from build123d import *

# Parameters (mm, degrees)
SKETCH_1_W             = 135
SKETCH_1_H             = 100
EXTRUDE_1_DEPTH        = 12
SKETCH_2_W             = 12.5
SKETCH_2_H             = 100
EXTRUDE_2_DEPTH        = 15
SKETCH_3_W             = 30
SKETCH_3_H             = 200
CUT_EXTRUDE_1_DEPTH    = 4
SKETCH_4_W             = 60
SKETCH_4_H             = 20
CUT_EXTRUDE_2_DEPTH    = 86.330240829
FILLET_1_R             = 5
HOLE_WIZARD_M6_1_D     = 5
HOLE_WIZARD_M6_1_DEPTH = 15
HOLE_WIZARD_M6_1_TIP   = 1.502151548
HOLE_WIZARD_M5_1_D     = 4.2
HOLE_WIZARD_M5_1_DEPTH = 12.4
HOLE_WIZARD_M5_1_TIP   = 1.2618073
CHAMFER_1_SIZE         = 0.5


with BuildPart() as part:
    # 草图1 → 凸台-拉伸1 (new body)
    with BuildSketch(Plane.XY):
        Rectangle(SKETCH_1_W, SKETCH_1_H)
    extrude(amount=EXTRUDE_1_DEPTH)

    # 草图2 → 凸台-拉伸2 (add)
    with BuildSketch(Plane.XY.offset(12)):
        with Locations((-61.25, 0)):
            Rectangle(SKETCH_2_W, SKETCH_2_H)
        with Locations((61.25, 0)):
            Rectangle(SKETCH_2_W, SKETCH_2_H)
    extrude(amount=EXTRUDE_2_DEPTH)

    # 草图3 → 切除-拉伸1 (cut)
    with BuildSketch(Plane.XY.offset(12)):
        with Locations((0, 50)):
            Rectangle(SKETCH_3_W, SKETCH_3_H)
    extrude(amount=-CUT_EXTRUDE_1_DEPTH, mode=Mode.SUBTRACT)

    # 草图4 → 切除-拉伸2 (cut, through all)
    with BuildSketch(Plane.XY.offset(12)):
        with Locations((0, 40)):
            Rectangle(SKETCH_4_W, SKETCH_4_H)
    extrude(amount=-CUT_EXTRUDE_2_DEPTH, mode=Mode.SUBTRACT)

    # 圆角1
    fillet_1_edges = [part.edges().sort_by_distance(p)[0] for p in [
        (30, 30, 6),
        (-30, 30, 6),
    ]]
    fillet(fillet_1_edges, radius=FILLET_1_R)

    # M6 螺纹孔1
    with Locations(Plane(origin=(0, 50, 0), x_dir=(1, 0, 0), z_dir=(0, 1, 0))):
        with Locations((-61.5, -21), (-47.5, -6), (47.5, -6), (61.5, -21)):
            Hole(HOLE_WIZARD_M6_1_D / 2, depth=HOLE_WIZARD_M6_1_DEPTH)
            with Locations((0, 0, -(HOLE_WIZARD_M6_1_DEPTH + HOLE_WIZARD_M6_1_TIP / 2))):  # 118° drill point
                Cone(0, HOLE_WIZARD_M6_1_D / 2, HOLE_WIZARD_M6_1_TIP, mode=Mode.SUBTRACT)

    # M5 螺纹孔1
    with Locations(Plane.XY.offset(27)):
        with Locations((-61.5, 30), (-61.5, -30), (61.5, -30), (61.5, 30)):
            Hole(HOLE_WIZARD_M5_1_D / 2, depth=HOLE_WIZARD_M5_1_DEPTH)
            with Locations((0, 0, -(HOLE_WIZARD_M5_1_DEPTH + HOLE_WIZARD_M5_1_TIP / 2))):  # 118° drill point
                Cone(0, HOLE_WIZARD_M5_1_D / 2, HOLE_WIZARD_M5_1_TIP, mode=Mode.SUBTRACT)

    # 倒角1
    chamfer_1_edges = [part.edges().sort_by_distance(p)[0] for p in [
        (-35, -50, 12),
        (-55, -50, 19.5),
        (-55, 50, 19.5),
        (-67.5, 0, 27),
        (-61.25, -50, 27),
        (-55, 0, 27),
        (-61.25, 50, 27),
        (42.5, 50, 12),
        (55, 50, 19.5),
        (55, -50, 19.5),
        (61.25, 50, 27),
        (55, 0, 27),
        (61.25, -50, 27),
        (67.5, 0, 27),
        (35, -50, 12),
        (0, -50, 0),
        (-67.5, 0, 0),
        (48.75, 50, 0),
        (67.5, 0, 0),
        (-48.75, 50, 0),
        (-42.5, 50, 12),
        (-30, 50, 6),
        (30, 50, 6),
        (67.5, -50, 13.5),
        (-67.5, -50, 13.5),
        (-67.5, 50, 13.5),
        (67.5, 50, 13.5),
    ]]
    chamfer(chamfer_1_edges, length=CHAMFER_1_SIZE)


solid = part.part
Design review of the part built by this model. Coordinates are the model's own, in mm. A direction names the side the tool comes from. Coordinates: 2 decimals unless noted, no trailing zeros. Loops run counter-clockwise (first coordinate to the right, second up) from the corner with the lowest first, then second, coordinate; pieces in that order, holes last.
Item 1: Wall thickness on L1, parallel to X at y = 30, z = 24; L2, parallel to Y at x = -61.5, z = 18.25; L3, parallel to X at y = 41.5, z = 21: over which ranges is each line inside the solid? List them lowest first.
Completed:
L1: x = -67.5 to -63.6, -59.4 to -55, 55 to 59.4, 63.6 to 67.5
L2: y = -50 to -32.1, -27.9 to 27.9, 32.1 to 50
L3: x = -67.5 to -64, -59 to -55, 55 to 59, 64 to 67.5
Item 2: Add section C-C (y = -34). Write out the cut boundary in (x, z).
Completed:
outline: (-67.5, 0.5) - (-67, 0) - (67, 0) - (67.5, 0.5) - (67.5, 26.5) - (67, 27) - (55.5, 27) - (55, 26.5) - (55, 12) - (15, 12) - (15, 8) - (-15, 8) - (-15, 12) - (-55, 12) - (-55, 26.5) - (-55.5, 27) - (-67, 27) - (-67.5, 26.5) - close
Item 3: Add section B-B (x = -17). Write out the cut boundary in (y, z).
Completed:
outline: (-50, 0.5) - (-49.5, 0) - (30, 0) - (30, 12) - (-49.5, 12) - (-50, 11.5) - close
Item 4: Draft analysis for pull direction X (two halves, no side actions). For faces 4 (the flat face through (67.5, -1, 13)), 5 (the cylindrical face through (-62.469, 28.137, 20.713)), 6 (the flat face through (53, 50, 10)), state which applies: pulls with the +X half, pulls with the -X half, needs draft (parallel to the pull), parting line crosses it, or undercut.
Completed:
face 4: pulls with the +X half
face 5: undercut
face 6: needs draft
Item 5: Add section A-A (y = 43). Write out the cut boundary in (x, z).
Completed:
outline: (-67.5, 0.5) - (-67, 0) - (-30, 0) - (-30, 12) - (-55, 12) - (-55, 26.5) - (-55.5, 27) - (-67, 27) - (-67.5, 26.5) - close; (30, 0) - (67, 0) - (67.5, 0.5) - (67.5, 26.5) - (67, 27) - (55.5, 27) - (55, 26.5) - (55, 12) - (30, 12) - close; hole circle Ø5 at (-61.5, 21); hole circle Ø5 at (-47.5, 6); hole circle Ø5 at (47.5, 6); hole circle Ø5 at (61.5, 21)
Item 6: Clearance check with flat-ended pins moving along their axes: pin 1 (20 mm diameter, centred on x = 41, y = -11, fed in from +Z); pin 2 (6 mm diameter, centred on x = -2.5, y = -28.5, fed in from +Z); pin 3 (9.5 mm diameter, centred on x = -0.5, z = 4, fed in from +Y). State where each tip first meets the part, or that it passes through.
Completed:
pin 1: stops at z = 12
pin 2: stops at z = 8
pin 3: stops at y = 30
Item 7: For faces 1 (the flat face through (35, 1, 12)), 2 (the flat face through (-30, 42, 6)), 3 (the cylindrical face through (-49.81, 42.4, 6.96)), list the 3-axis set-ups (+Z, -Z, +X, -X, +Y, -Y) from which the entire face can be reached by the end or side of a thin tool; tool diameter is ignored.
Completed:
face 1: +Z, +Y, -Y
face 2: +Z, -Z, +Y
face 3: +Y
